from build123d import *

# Parameters (mm, degrees)
EXTRUDE_1_DEPTH     = 7
FILLET_1_R          = 3
CUT_EXTRUDE_1_REACH = 177.71
SKETCH_3_R          = 3.5
CUT_EXTRUDE_2_REACH = 192.252
SKETCH_4_R          = 3.5


with BuildPart() as part:
    # 草图1 → 凸台-拉伸1 (new, symmetric)
    with BuildSketch(Plane.XY):
        Polygon((0, 180), (-15, 180), (-15, 15), (-60, 15), (-60, 0), (0, 0), align=None)
    extrude(amount=EXTRUDE_1_DEPTH, both=True)

    # 圆角1
    fillet_1_edges = [part.edges().sort_by_distance(p)[0] for p in [
        (-15, 15, 0),
    ]]
    fillet(fillet_1_edges, radius=FILLET_1_R)

    # 草图3 → 切除-拉伸1 (cut, up to next)
    with BuildSketch(Plane(origin=(0, 15, 0), x_dir=(1, 0, 0), z_dir=(0, 1, 0)), mode=Mode.PRIVATE) as cut_extrude_1_sk1:
        with Locations(Location((-52, 0, 0), (0, 0, 180))):
            Circle(SKETCH_3_R)
    cut_extrude_1_tool1 = extrude(cut_extrude_1_sk1.sketch, amount=-CUT_EXTRUDE_1_REACH, mode=Mode.PRIVATE) & part.part
    # 草图3 → 切除-拉伸1 (cut, up to next)
    with BuildSketch(Plane(origin=(0, 15, 0), x_dir=(1, 0, 0), z_dir=(0, 1, 0)), mode=Mode.PRIVATE) as cut_extrude_1_sk2:
        with Locations(Location((-30, 0, 0), (0, 0, 180))):
            Circle(SKETCH_3_R)
    cut_extrude_1_tool2 = extrude(cut_extrude_1_sk2.sketch, amount=-CUT_EXTRUDE_1_REACH, mode=Mode.PRIVATE) & part.part
    add(cut_extrude_1_tool1.solids().sort_by_distance((-52, 15, 0))[0], mode=Mode.SUBTRACT)
    add(cut_extrude_1_tool2.solids().sort_by_distance((-30, 15, 0))[0], mode=Mode.SUBTRACT)

    # 草图4 → 切除-拉伸2 (cut, up to next)
    with BuildSketch(Plane(origin=(0, 0, -7), x_dir=(-1, 0, 0), z_dir=(0, 0, -1)), mode=Mode.PRIVATE) as cut_extrude_2_sk1:
        with Locations((7, 146.5)):
            Circle(SKETCH_4_R)
    cut_extrude_2_tool1 = extrude(cut_extrude_2_sk1.sketch, amount=-CUT_EXTRUDE_2_REACH, mode=Mode.PRIVATE) & part.part
    add(cut_extrude_2_tool1.solids().sort_by_distance((-7, 146.5, -7))[0], mode=Mode.SUBTRACT)


solid = part.part
Can you work these out from the model? Positions are in its coordinate system, mm. A direction names the side the tool comes from. Coordinates: 2 decimals unless noted, no trailing zeros. Write each loop counter-clockwise with the first axis right and the second up, starting at its lowest first coordinate (ties: lowest second). Pieces come first, ordered by that corner, then holes.
Q1. Which directions (+Z, -Z, +X, -X, +Y, -Y) give clear straight access to the entire face, cutting with the end or side of a thin tool? Please do faces 1 (the face through (-39, 15, 0)), 2 (the face through (-30, 0, 5)).
Results found:
face 1: +Z, -Z, -X, +Y
face 2: +Z, -Z, +X, -X, -Y
Q2. Imagine slicing it at C-C, the plane y = 146.5. List the corners of the cut face in (x, z) for me, plus the area to 3 significant figures.
Results found:
outline: (-15, -7) - (-10.5, -7) - (-10.5, 7) - (-15, 7) - close; (-3.5, -7) - (0, -7) - (0, 7) - (-3.5, 7) - close
area: 112 mm2
Q3. Imagine slicing it at B-B, the plane x = -7. List the corners of the cut face in (y, z) for me, plus the area to 3 significant figures.
Results found:
outline: (0, -7) - (143, -7) - (143, 7) - (0, 7) - close; (150, -7) - (180, -7) - (180, 7) - (150, 7) - close
area: 2,420 mm2
Q4. For P1, Ø4, axis at y = 102.5, z = 3, coming from the -X side; P2, Ø5, axis at x = -34.5, z = 0, coming from the +Y side, each with a flat end and sliding along its axis, tell me the tip position at first contact or that it passes through.
Results found:
P1: stops at x = -15
P2: stops at y = 15
Q5. Imagine slicing it at D-D, the plane y = 32. List the corners of the cut face in (x, z) for me, plus the area to 3 significant figures.
Results found:
outline: (-15, -7) - (0, -7) - (0, 7) - (-15, 7) - close
area: 210 mm2
Q6. Please list where these lines run through material, in increasing order: L1, parallel to Z at x = -52, y = 12; L2, parallel to X at y = 159, z = -3; L3, parallel to Y at x = -7, z = 3.
Results found:
L1: z = -7 to -3.5, 3.5 to 7
L2: x = -15 to 0
L3: y = 0 to 143, 150 to 180
Q7. Imagine slicing it at A-A, the plane z = 0. List the corners of the cut face in (x, y) for me, plus the area to 3 significant figures.
Results found:
outline: (-60, 0) - (-55.5, 0) - (-55.5, 15) - (-60, 15) - close; (-48.5, 0) - (-33.5, 0) - (-33.5, 15) - (-48.5, 15) - close; (-26.5, 0) - (0, 0) - (0, 180) - (-15, 180) - (-15, 18) arc R3 cw to (-18, 15) - (-26.5, 15) - close; hole circle Ø7 at (-7, 146.5)
area: 3,130 mm2
Q8. If we mould it in two halves opening along X, with no side actions, what happens to faces 3 (the face through (-15.9, 15.86, 0.1)), 4 (the face through (0, 89, 0)), 5 (the face through (-33.34, 7.6, 1.05))? For each: +X half, -X half, draft (parallel to the pull), parting line (faces both ways), or undercut.
Results found:
face 3: -X half
face 4: +X half
face 5: undercut
